from build123d import *

# Parameters (mm, degrees)
BOSS_EXTRUDE1_DEPTH = 20
SKETCH2_R           = 10
CUT_EXTRUDE1_DEPTH  = 79.74007874
SKETCH3_W           = 35
SKETCH3_H           = 60
BOSS_EXTRUDE5_DEPTH = 15


with BuildPart() as part:
    # Sketch1 → Boss-Extrude1 (new body)
    with BuildSketch(Plane.XY):
        with BuildLine():
            Line((-40, 30), (40, 30))
            Line((40, 30), (40, -30))
            Line((40, -30), (-40, -30))
            ThreePointArc((-40, -30), (-70, 0), (-40, 30))
        make_face()
    extrude(amount=BOSS_EXTRUDE1_DEPTH)

    # Sketch2 → Cut-Extrude1 (cut, through all)
    with BuildSketch(Plane(origin=(0, 0, 0), x_dir=(-1, 0, 0), z_dir=(0, 0, -1))):
        with Locations((40, 0)):
            Circle(SKETCH2_R)
    extrude(amount=-CUT_EXTRUDE1_DEPTH, mode=Mode.SUBTRACT)

    # Sketch3 → Boss-Extrude5 (add)
    with BuildSketch(Plane(origin=(40, 0, 0), x_dir=(0, 0, -1), z_dir=(1, 0, 0))):
        with Locations((-2.5, 0)):
            Rectangle(SKETCH3_W, SKETCH3_H)
    extrude(amount=BOSS_EXTRUDE5_DEPTH)

    # Mirror1: part across plane


with BuildPart() as part_1:
    add(part.part)
    add(part.part.mirror(Plane(origin=(55, -30, -15), x_dir=(1, 0, 0), z_dir=(0, 0, 1))))


solid = part_1.part
Geometry: final body of the model. Coordinates: model frame, mm. A direction names the side the tool comes from. Round coordinates to 2 decimals unless told otherwise and drop trailing zeros. Order: outer loops, then holes, each group sorted by start corner. A loop starts at its lowest first (then second) coordinate and runs counter-clockwise, first axis right, second up.
Q1. Mould query, pull axis Z, two halves, no side actions, for faces 3 (the face through (-8, 0, 20)), 4 (the face through (-69.993, -0.66, -39.86)), 5 (the face through (40, 0, -15)). Classes: released by +Z, released by -Z, zero draft, split by the parting line, or undercut.
Result sheet:
face 3: released by +Z
face 4: zero draft
face 5: undercut
Q2. Access query for faces 1 (the face through (7, 30, -31)), 2 (the face through (-14, 0, -30)). Directions: +Z, -Z, +X, -X, +Y, -Y. A direction counts if a zero-diameter tool reaches every point of the face in a straight line with its end or side. Return the directions, or none.
Result sheet:
face 1: +Z, -Z, +X, -X, +Y
face 2: -X, +Y, -Y
Q3. Section A-A, the plane x = 30.5. Output: boundary loops of the cut face in (y, z).
Result sheet:
outline: (-30, -50) - (30, -50) - (30, -30) - (-30, -30) - close; (-30, 0) - (30, 0) - (30, 20) - (-30, 20) - close
Q4. Section B-B, the plane y = 0. Output: boundary loops of the cut face in (x, z).
Result sheet:
outline: (-70, -50) - (-50, -50) - (-50, -30) - (-70, -30) - close; (-70, 0) - (-50, 0) - (-50, 20) - (-70, 20) - close; (-30, -50) - (55, -50) - (55, 20) - (-30, 20) - (-30, 0) - (40, 0) - (40, -30) - (-30, -30) - close
Q5. Section C-C, the plane x = -36.5. Output: boundary loops of the cut face in (y, z).
Result sheet:
outline: (-30, -50) - (-9.37, -50) - (-9.37, -30) - (-30, -30) - close; (-30, 0) - (-9.37, 0) - (-9.37, 20) - (-30, 20) - close; (9.37, -50) - (30, -50) - (30, -30) - (9.37, -30) - close; (9.37, 0) - (30, 0) - (30, 20) - (9.37, 20) - close
Q6. Pin query (flat end, axial travel): pin 1 (4 mm diameter, centred on y = 10, z = -13.5, fed in from -X). Return the tip coordinate at first contact, or that it passes through.
Result sheet:
pin 1: stops at x = 40
Q7. Material intervals for probe 1 along Z at (x, y) = (39, 2.5); probe 2 along Y at (x, z) = (-40, -42); probe 3 along X at (y, z) = (2.5, 15.5), sorted ascending.
Result sheet:
probe 1: z = -50 to -30, 0 to 20
probe 2: y = -30 to -10, 10 to 30
probe 3: x = -69.9 to -49.68, -30.32 to 55
Q8. Section D-D, the plane z = 3. Output: boundary loops of the cut face in (x, y).
Result sheet:
outline: (-40, -30) - (55, -30) - (55, 30) - (-40, 30) arc R30 ccw to start; hole circle Ø20 at (-40, 0)
